Geometry: final body of the model. Coordinates: model frame, mm. A direction names the side the tool comes from. Coordinates: 2 decimals unless noted, no trailing zeros. Order: outer loops, then holes, each group sorted by start corner. A loop starts at its lowest first (then second) coordinate and runs counter-clockwise, first axis right, second up. Notation, with made-up numbers: M -17,-32.75 L 36,-32.75 A25 ccw 36,0.25 Z; hole C 38.25,-30.75 d8. An arc over 180 degrees is marked long. Use CSV: the item, a comma, the result in double quotes. Start each with the question number.
Q1. Mould query, pull axis Z, two halves, no side actions, for faces 4 (the face through (-26.25, 3, 14.58)), 5 (the face through (-31.64, 0.07, 31.1)), 6 (the face through (-29, -5, 16)). Classes: +Z half, -Z half, draft (parallel to the pull), parting line (faces both ways), or undercut.
Q2. Section query C-C, the plane y = 2.25. Output: boundary loops of the cut face in (x, z), and give its area (3 significant figures).
Q3. Section query A-A, the plane z = 6.5. Output: boundary loops of the cut face in (x, y), and give its area (3 significant figures).
Q4. Section query D-D, the plane z = 27. Output: boundary loops of the cut face in (x, y).
Q5. First-contact query: P1, Ø4, axis at x = -11, z = 5, coming from the +Y side; P2, Ø3, axis at x = 24, z = 16.5, coming from the -Y side; P3, Ø7, axis at x = -25, z = 16, coming from the +Y side; P4, Ø1.8, axis at x = -25.5, z = 15.5, coming from the -Y side. Flat tips, straight axial feed; report the tip coordinate or a pass-through.
Q6. Access query for faces 1 (the face through (23.198, 4.014, 10.277)), 2 (the face through (0, 5, 16)), 3 (the face through (0, -3, 16)). Directions: +Z, -Z, +X, -X, +Y, -Y. A direction counts if a zero-diameter tool reaches every point of the face in a straight line with its end or side. Return the directions, or none.
Q7. Section query B-B, the plane x = -12. Output: boundary loops of the cut face in (y, z).
Q8. Ray query, probe 1 along X at (y, z) = (1, 16); probe 2 along X at (y, z) = (3.55, 16); probe 3 along Z at (x, y) = (-25, -3.5). Return the intervals inside material, ascending.
from build123d import *

# Parameters (mm, degrees)
SKETCH_1_W                = 65
SKETCH_1_H                = 10
EXTRUDE_1_DEPTH           = 32
HOLE_WIZARD_5_0_5_1_D     = 4.3
FILLET_1_R                = 3
SKETCH_10_R               = 6
CUT_EXTRUDE_3_DEPTH       = 2
HOLE_WIZARD_1_D           = 3.4
HOLE_WIZARD_1_CBORE_D     = 6
HOLE_WIZARD_1_CBORE_DEPTH = 3.4
HOLE_WIZARD_2_D           = 4.3
HOLE_WIZARD_2_CBORE_D     = 8
HOLE_WIZARD_2_CBORE_DEPTH = 4.6
SKETCH_16_W               = 39.2
SKETCH_16_H               = 72.88385863
CUT_EXTRUDE_4_DEPTH       = 2


with BuildPart() as part:
    # 草图1 → 凸台-拉伸1 (new body)
    with BuildSketch(Plane.XY):
        Rectangle(SKETCH_1_W, SKETCH_1_H)
    extrude(amount=EXTRUDE_1_DEPTH)

    # Ø5.0 (5) 直径孔1 (through all)
    with Locations(Plane.XZ.offset(5)):
        with Locations((-12, 6.5), (12, 6.5)):
            Hole(HOLE_WIZARD_5_0_5_1_D / 2)

    # 圆角1
    fillet_1_edges = [part.edges().sort_by_distance(p)[0] for p in [
        (-32.5, 0, 32),
        (32.5, 0, 32),
        (-32.5, 0, 0),
        (32.5, 0, 0),
    ]]
    fillet(fillet_1_edges, radius=FILLET_1_R)

    # 草图10 → 切除-拉伸3 (cut)
    with BuildSketch(Plane(origin=(0, 5, 0), x_dir=(1, 0, 0), z_dir=(0, 1, 0))):
        with Locations(Location((-25, -16, 0), (0, 0, 270))):
            Circle(SKETCH_10_R)
        with Locations(Location((25, -16, 0), (0, 0, 90))):
            Circle(SKETCH_10_R)
    extrude(amount=-CUT_EXTRUDE_3_DEPTH, mode=Mode.SUBTRACT)

    # 打孔尺寸(%根据)开槽圆柱头螺钉的类型1 (through all)
    with Locations(Plane(origin=(0, -5, 0), x_dir=(-1, 0, 0), z_dir=(0, -1, 0))):
        with Locations((-25, -16), (25, -16)):
            CounterBoreHole(HOLE_WIZARD_1_D / 2, HOLE_WIZARD_1_CBORE_D / 2, HOLE_WIZARD_1_CBORE_DEPTH)

    # 打孔尺寸(%根据)开槽圆柱头螺钉的类型2 (through all)
    with Locations(Plane(origin=(0, 5, 0), x_dir=(1, 0, 0), z_dir=(0, 1, 0))):
        with Locations((-12, -6.5), (12, -6.5)):
            CounterBoreHole(HOLE_WIZARD_2_D / 2, HOLE_WIZARD_2_CBORE_D / 2, HOLE_WIZARD_2_CBORE_DEPTH)

    # 草图16 → 切除-拉伸4 (cut)
    with BuildSketch(Plane.XZ.offset(5)):
        Rectangle(SKETCH_16_W, SKETCH_16_H)
    extrude(amount=-CUT_EXTRUDE_4_DEPTH, mode=Mode.SUBTRACT)


solid = part.part
Responses:
1,face 4,"undercut"
1,face 5,"+Z half"
1,face 6,"draft"
2,outline,"M -32.5,3 A3 ccw -29.5,0 L 29.5,0 A3 ccw 32.5,3 L 32.5,29 A3 ccw 29.5,32 L -29.5,32 A3 ccw -32.5,29 Z; hole C -25,16 d3.4; hole C -12,6.5 d8; hole C 12,6.5 d8; hole C 25,16 d3.4"
2,area,"1,950 mm²"
3,outline,"M -32.5,-5 L -19.6,-5 L -19.6,-3 L -14.15,-3 L -14.15,0.4 L -16,0.4 L -16,5 L -32.5,5 Z; M -9.85,-3 L 9.85,-3 L 9.85,0.4 L 8,0.4 L 8,5 L -8,5 L -8,0.4 L -9.85,0.4 Z; M 14.15,-3 L 19.6,-3 L 19.6,-5 L 32.5,-5 L 32.5,5 L 16,5 L 16,0.4 L 14.15,0.4 Z"
3,area,"469 mm²"
4,outline,"M -32.5,-5 L -19.6,-5 L -19.6,-3 L 19.6,-3 L 19.6,-5 L 32.5,-5 L 32.5,5 L -32.5,5 Z"
5,P1,"stops at y = 0.4"
5,P2,"stops at y = -1.6"
5,P3,"stops at y = 3"
5,P4,"passes through"
6,face 1,"+Y"
6,face 2,"+Z, -Z, +X, -X, +Y"
6,face 3,"+Z, -Z, -Y"
7,outline,"M -3,0 L 5,0 L 5,2.5 L 0.4,2.5 L 0.4,4.35 L -3,4.35 Z; M -3,8.65 L 0.4,8.65 L 0.4,10.5 L 5,10.5 L 5,32 L -3,32 Z"
8,probe 1,"x = -32.5 to -26.7, -23.3 to 23.3, 26.7 to 32.5"
8,probe 2,"x = -32.5 to -31, -19 to 19, 31 to 32.5"
8,probe 3,"z = 0 to 13, 19 to 32"
